The listing builds one solid part. Answer for the finished solid, in the listing's coordinates (mm). Give positions to 0.01 mm unless a question says otherwise; leave off trailing zeros. Loops run counter-clockwise (first coordinate to the right, second up) from the corner with the lowest first, then second, coordinate; pieces in that order, holes last.
Item 1: The mould has two halves that part along X. Classify faces 1 (the face through (25.652, 0.275, 4.93)), 2 (the face through (-25.652, -0.275, 4.93)), 3 (the face through (0, -12.5, 5)), 4 (the face through (-8.54, -1.92, 4.93)): pulls with the +X half, pulls with the -X half, needs draft (parallel to the pull), parting line crosses it, or undercut.
Item 2: Section D-D, the plane y = 5.75 is taken. Give the vertices of the cut face in (x, z), and give its area (3 significant figures).
Item 3: Section C-C, the plane x = -11.5 is taken. Give the vertices of the cut face in (y, z).
Item 4: Section A-A, the plane y = 0 is taken. Give the vertices of the cut face in (x, z) (3 decimals).
Item 5: Section B-B, the plane z = 5 is taken. Give the vertices of the cut face in (x, y) (3 decimals).
Item 6: Consider line 1 along Y through (x, z) = (-13, 7.5); line 2 along X through (y, z) = (1.5, 8.5); line 3 along X through (y, z) = (0.5, 1.25) (3 decimals). Determine where each line is inside the solid, lowest interval first.
Item 7: Each of these flat-tipped pins is pushed along its axis until it touches: pin 1 Ø10 at (x, y) = (7.5, 1.5) entering from -Z; pin 2 Ø1 at (x, y) = (19, -3.5) entering from +Z; pin 3 Ø3 at (y, z) = (7.5, 1.5) entering from +X. Where does it stop, or does it pass through?
from build123d import *

# Parameters (mm, degrees)
SKETCH_1_R      = 7.5
SKETCH_1_R_2    = 5
EXTRUDE_1_DEPTH = 10


with BuildPart() as part:
    # 草图1 → 凸台-拉伸1 (new body)
    with BuildSketch(Plane.XY):
        with BuildLine():
            Line((-13.155, 12.5), (13.155, 12.5))
            ThreePointArc((13.155, 12.5), (25.655, 0), (13.155, -12.5))
            Line((13.155, -12.5), (-13.155, -12.5))
            ThreePointArc((-13.155, -12.5), (-25.655, 0), (-13.155, 12.5))
        make_face()
        with Locations((13.155, 0)):
            Circle(SKETCH_1_R, mode=Mode.SUBTRACT)
        with Locations((-13.155, 0)):
            Circle(SKETCH_1_R_2, mode=Mode.SUBTRACT)
    extrude(amount=EXTRUDE_1_DEPTH)


solid = part.part
Worked answers:
1. face 1: pulls with the +X half
1. face 2: pulls with the -X half
1. face 3: needs draft
1. face 4: undercut
2. outline: (-24.25, 0) - (8.34, 0) - (8.34, 10) - (-24.25, 10) - close; (17.97, 0) - (24.25, 0) - (24.25, 10) - (17.97, 10) - close
2. area: 389 mm2
3. outline: (-12.5, 0) - (-4.72, 0) - (-4.72, 10) - (-12.5, 10) - close; (4.72, 0) - (12.5, 0) - (12.5, 10) - (4.72, 10) - close
4. outline: (-25.655, 0) - (-18.155, 0) - (-18.155, 10) - (-25.655, 10) - close; (-8.155, 0) - (5.655, 0) - (5.655, 10) - (-8.155, 10) - close; (20.655, 0) - (25.655, 0) - (25.655, 10) - (20.655, 10) - close
5. outline: (-13.155, -12.5) - (13.155, -12.5) arc R12.5 ccw to (13.155, 12.5) - (-13.155, 12.5) arc R12.5 ccw to start; hole circle Ø10 at (-13.155, 0); hole circle Ø15 at (13.155, 0)
6. line 1: y = -12.5 to -5, 5 to 12.5
6. line 2: x = -25.56 to -17.92, -8.39 to 5.81, 20.5 to 25.56
6. line 3: x = -25.645 to -18.13, -8.18 to 5.672, 20.638 to 25.645
7. pin 1: stops at z = 0
7. pin 2: passes through
7. pin 3: stops at x = 24.12
